```python
from build123d import *

# Parameters (mm, degrees)
BASE_PLATE_DEPTH       = 25
BASE_SLOT_DEPTH        = 50
UPRIGHT_BLOCK_SKETCH_W = 72
UPRIGHT_BLOCK_SKETCH_H = 36
UPRIGHT_BLOCK_DEPTH    = 65
BEARING_SEAT_CUT_DEPTH = 12
THROUGH_BORE_SKETCH_R  = 12
THROUGH_BORE_DEPTH     = 106


with BuildPart() as part:
    # Base Plate Sketch → Base Plate (new body)
    with BuildSketch(Plane(origin=(0, 0, 0), x_dir=(1, 0, 0), z_dir=(0, 1, 0))):
        Polygon((36, 0), (36, 72.5), (-36, 72.5), (-36, -72.5), (36, -72.5), align=None)
    extrude(amount=BASE_PLATE_DEPTH)

    # Base Slot Sketch → Base Slot (cut)
    with BuildSketch(Plane(origin=(0, 25, 0), x_dir=(1, 0, 0), z_dir=(0, 1, 0))):
        with BuildLine():
            Line((12, 22.5), (12, 72.5))
            Line((12, 72.5), (-12, 72.5))
            Line((-12, 72.5), (-12, 22.5))
            ThreePointArc((-12, 22.5), (0, 10.5), (12, 22.5))
        make_face()
    extrude(amount=-BASE_SLOT_DEPTH, mode=Mode.SUBTRACT)

    # Upright Block Sketch → Upright Block (add)
    with BuildSketch(Plane(origin=(0, 25, 0), x_dir=(1, 0, 0), z_dir=(0, 1, 0))):
        with Locations((0, -54.5)):
            Rectangle(UPRIGHT_BLOCK_SKETCH_W, UPRIGHT_BLOCK_SKETCH_H)
    extrude(amount=UPRIGHT_BLOCK_DEPTH)

    # Bearing Seat Sketch → Bearing Seat Cut (cut)
    with BuildSketch(Plane.XY.offset(72.5)):
        with BuildLine():
            Line((-36, 66), (-36, 30))
            Line((-36, 30), (-24, 30))
            ThreePointArc((-24, 30), (0, 18), (24, 30))
            Line((24, 30), (36, 30))
            Line((36, 30), (36, 66))
            Line((36, 66), (24, 66))
            ThreePointArc((24, 66), (0, 78), (-24, 66))
            Line((-24, 66), (-36, 66))
        make_face()
    extrude(amount=-BEARING_SEAT_CUT_DEPTH, mode=Mode.SUBTRACT)

    # Through Bore Sketch → Through Bore (cut)
    with BuildSketch(Plane.XY.offset(60.5)):
        with Locations((0, 48)):
            Circle(THROUGH_BORE_SKETCH_R)
    extrude(amount=-THROUGH_BORE_DEPTH, mode=Mode.SUBTRACT)


solid = part.part
```
The listing builds one solid part. Answer for the finished solid, in the listing's coordinates (mm). A direction names the side the tool comes from. Round coordinates to 2 decimals unless told otherwise and drop trailing zeros. Order: outer loops, then holes, each group sorted by start corner. A loop starts at its lowest first (then second) coordinate and runs counter-clockwise, first axis right, second up. Notation, with made-up numbers: (-17, 69.5) -> (31, 69.5) arc R30 cw to (31, 107.5) -> close; hole circle Ø2 at (50, 64). An arc over 180 degrees is marked (long way). Answer as CSV lines item,"result". Start each with the question number.
(1) A tool of negligible diameter and unlimited length cuts with its end or side. For faces 1 (the face through (30, 30, 67)), 2 (the face through (-1, 25, -7)), 3 (the face through (-36, 24, 17)), 4 (the face through (-1, 62, 60.5)), 5 (the face through (-12, 13, -48)), from which of +Z, -Z, +X, -X, +Y, -Y can it reach the whole face along a straight path? Write none if from no direction.
(2) The part is cut by section C-C (y = 48). Determine the outline of the cut face in (x, z).
(3) The part is cut by section D-D (x = 27.5). Determine the outline of the cut face in (y, z).
(4) Find the intervals of material crossed by probe 1 along X at (y, z) = (8, -55.5); probe 2 along Y at (x, z) = (0, 52); probe 3 along Z at (x, y) = (-31, 43), in increasing order. Write a range as from..to.
(5) The part is cut by section A-A (z = -39.5). Determine the outline of the cut face in (x, y).
(6) The part is cut by section B-B (x = 0). Determine the outline of the cut face in (y, z).
(7) For a pull along Y with two mould halves and no side action, classify faces 6 (the face through (-30, 30, 67)), 7 (the face through (-1, 0, -1)), 8 (the face through (36, 24, 17)) as +Y half, -Y half, draft (parallel to the pull), parting line (faces both ways), or undercut.
(8) Flat-ended cylindrical pins translate along their axes: pin 1 Ø4 at (x, y) = (3.5, 74.5) entering from -Z; pin 2 Ø12 at (x, y) = (1, 15) entering from -Z; pin 3 Ø6 at (x, y) = (-21.5, 34) entering from +Z. Find the tip coordinate at first contact, or state that the pin passes through.
Evaluation:
1,face 1,"+Z, +X, -X"
1,face 2,"-Z, +X, -X, +Y"
1,face 3,"+Z, -Z, -X, +Y, -Y"
1,face 4,"+Z"
1,face 5,"-Z, +Y, -Y"
2,outline,"(-36, 36.5) -> (-12, 36.5) -> (-12, 60.5) -> (-36, 60.5) -> close; (12, 36.5) -> (36, 36.5) -> (36, 60.5) -> (12, 60.5) -> close"
3,outline,"(0, -72.5) -> (25, -72.5) -> (25, 36.5) -> (90, 36.5) -> (90, 72.5) -> (66, 72.5) -> (66, 60.5) -> (30, 60.5) -> (30, 72.5) -> (0, 72.5) -> close"
4,probe 1,"-36..-12, 12..36"
4,probe 2,"0..36, 60..90"
4,probe 3,"36.5..60.5"
5,outline,"(-36, 0) -> (-12, 0) -> (-12, 25) -> (-36, 25) -> close; (12, 0) -> (36, 0) -> (36, 25) -> (12, 25) -> close"
6,outline,"(0, -10.5) -> (25, -10.5) -> (25, 36.5) -> (36, 36.5) -> (36, 60.5) -> (18, 60.5) -> (18, 72.5) -> (0, 72.5) -> close; (60, 36.5) -> (90, 36.5) -> (90, 72.5) -> (78, 72.5) -> (78, 60.5) -> (60, 60.5) -> close"
7,face 6,"undercut"
7,face 7,"-Y half"
7,face 8,"draft"
8,pin 1,"z = 36.5"
8,pin 2,"z = -12.75"
8,pin 3,"z = 60.5"
